For this review, use the dimensioned drawing (mm, ordinates from the lowest corner) and the shaded views. Coordinates: 2 decimals unless noted, no trailing zeros. Loops run counter-clockwise (first coordinate to the right, second up) from the corner with the lowest first, then second, coordinate; pieces in that order, holes last.
1. To check wall thickness, follow probe 1 along X at (y, z) = (1.8, 33.5) (1 decimal); probe 2 along Z at (x, y) = (45.5, 0.7) (1 decimal); probe 3 along X at (y, z) = (1.55, 10) (1 decimal). State the ranges of each line that lie inside material, in increasing order.
2. Take a section at B-B, the plane y = 0.75. Count the separate pieces of the cut face and the enclosed holes in it, then the cut area to 3 significant figures.
3. Take a section at A-A, the plane z = 15. State the section outline as (x, y) points.
4. Take a section at D-D, the plane x = 28.1. State the section outline as (y, z) points.
5. Take a section at C-C, the plane x = 41. State the section outline as (y, z) points.
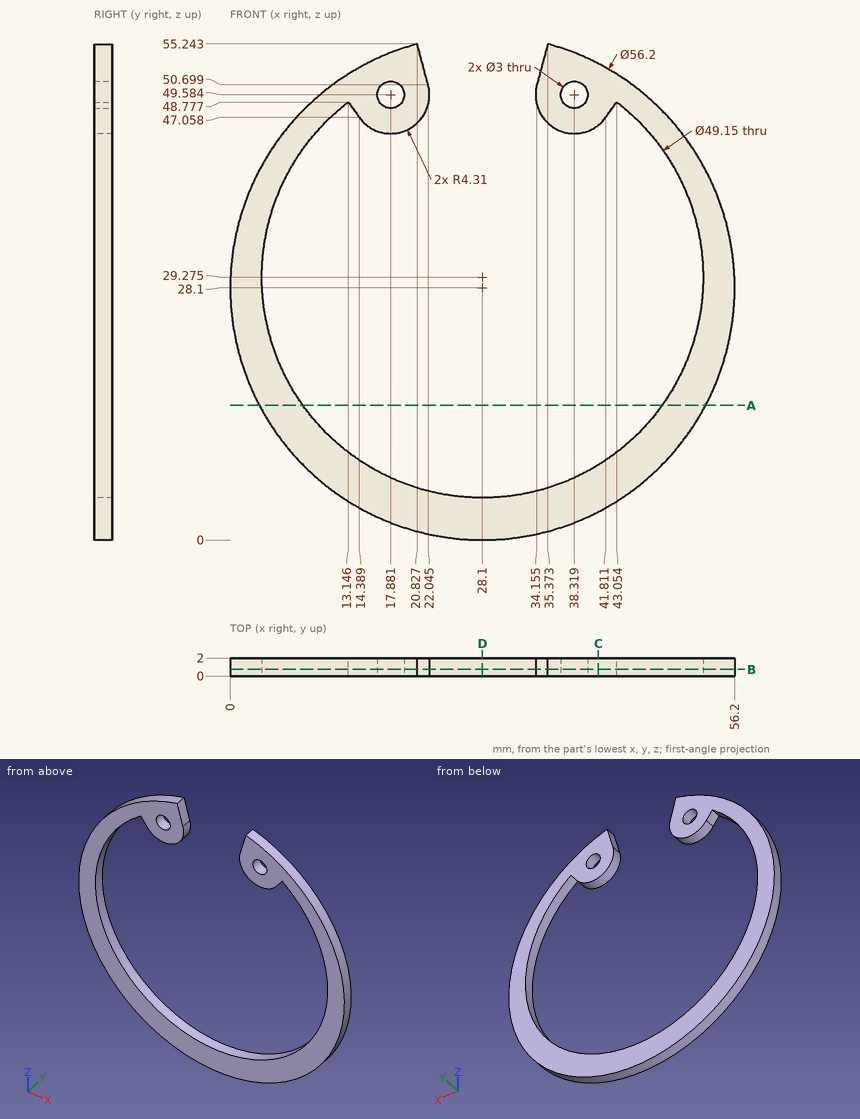
Results list:
1. probe 1: x = 0.5 to 3.9, 52.3 to 55.7
1. probe 2: z = 6 to 11.9, 46.6 to 50.2
1. probe 3: x = 6.6 to 12.9, 43.3 to 49.6
2. separate pieces: 1
2. enclosed holes: 2
2. area: 625 mm2
3. outline: (3.24, 0) - (8.1, 0) - (8.1, 2) - (3.24, 2) - close; (48.1, 0) - (52.96, 0) - (52.96, 2) - (48.1, 2) - close
4. outline: (0, 0) - (2, 0) - (2, 4.7) - (0, 4.7) - close
5. outline: (0, 3.14) - (2, 3.14) - (2, 8.36) - (0, 8.36) - close; (0, 46.21) - (2, 46.21) - (2, 53.06) - (0, 53.06) - close
